For this review, use the dimensioned drawing (mm, ordinates from the lowest corner) and the shaded views. A direction names the side the tool comes from. Round coordinates to 2 decimals unless told otherwise and drop trailing zeros. Loops run counter-clockwise (first coordinate to the right, second up) from the corner with the lowest first, then second, coordinate; pieces in that order, holes last.
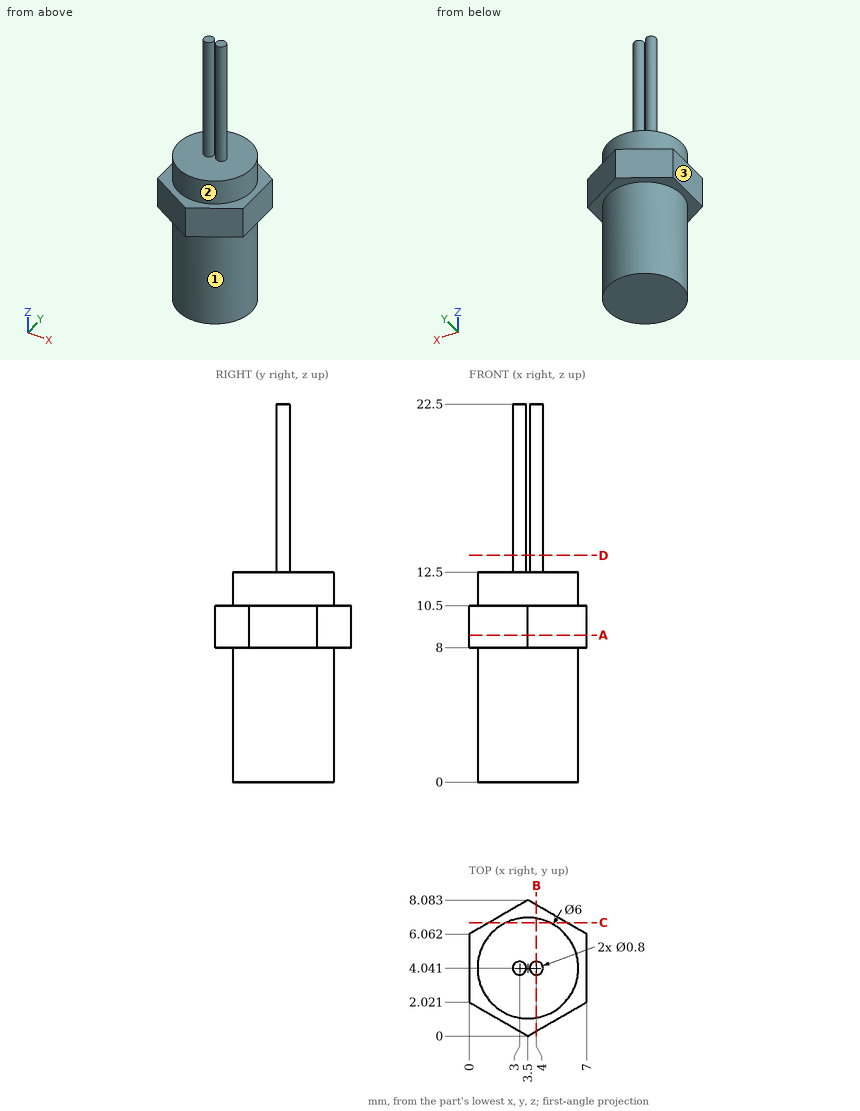
(1) For L1, parallel to Z at x = 5.5, y = 5; L2, parallel to X at y = 4, z = 4; L3, parallel to Z at x = 5, y = 6.75, list the stretches that pass through material, from the lowest coordinate up.
(2) Add section A-A (z = 8.75). Give the boundary of the cut face in (x, y).
(3) For the marked faces 1, 2 and 3, list the 3-axis set-ups (+Z, -Z, +X, -X, +Y, -Y) from which the entire face can be reached by the end or side of a thin tool; tool diameter is ignored.
(4) Add section C-C (y = 6.75). Give the boundary of the cut face in (x, z).
(5) Insertion check: pin 1 Ø2 at (x, z) = (6, 8.5) entering from +Y; pin 2 Ø2 at (x, y) = (2.5, 6.5) entering from +Z. Each pin has a flat end and moves straight along its axis. Give the tip position at first contact, or say it passes through.
(6) Add section B-B (x = 4). Give the boundary of the cut face in (y, z) (1 decimal).
(7) Add section D-D (z = 13.5). Give the boundary of the cut face in (x, y).
Outcome:
1. L1: z = 0 to 12.5
1. L2: x = 0.5 to 6.5
1. L3: z = 8 to 10.5
2. outline: (0, 2.02) - (3.5, 0) - (7, 2.02) - (7, 6.06) - (3.5, 8.08) - (0, 6.06) - close
3. face 1: -Z
3. face 2: +Z
3. face 3: +Z, -Z, -X, +Y, -Y
4. outline: (1.19, 8) - (2.21, 8) - (2.21, 0) - (4.79, 0) - (4.79, 8) - (5.81, 8) - (5.81, 10.5) - (4.79, 10.5) - (4.79, 12.5) - (2.21, 12.5) - (2.21, 10.5) - (1.19, 10.5) - close
5. pin 1: stops at y = 7.22
5. pin 2: stops at z = 12.5
6. outline: (0.3, 8) - (1.1, 8) - (1.1, 0) - (7, 0) - (7, 8) - (7.8, 8) - (7.8, 10.5) - (7, 10.5) - (7, 12.5) - (4.4, 12.5) - (4.4, 22.5) - (3.6, 22.5) - (3.6, 12.5) - (1.1, 12.5) - (1.1, 10.5) - (0.3, 10.5) - close
7. outline: circle Ø0.8 at (3, 4.04); circle Ø0.8 at (4, 4.04)
